Model file for the job. Use its own axes, mm. Face numbers are marked on the shaded views. A direction names the side the tool comes from. Coordinates: 2 decimals unless noted, no trailing zeros. Order: outer loops, then holes, each group sorted by start corner. A loop starts at its lowest first (then second) coordinate and runs counter-clockwise, first axis right, second up.
from build123d import *

# Parameters (mm, degrees)
SKETCH1_W           = 72
SKETCH1_H           = 26
BOSS_EXTRUDE1_DEPTH = 16
SKETCH2_W           = 40
SKETCH2_H           = 26
BOSS_EXTRUDE2_DEPTH = 69
SKETCH3_R           = 3.5
SKETCH3_R_2         = 3
CUT_EXTRUDE1_DEPTH  = 96.5
SKETCH4_R           = 6
CUT_EXTRUDE2_DEPTH  = 6
SKETCH5_R           = 2.5
CUT_EXTRUDE3_DEPTH  = 15


with BuildPart() as part:
    # Sketch1 → Boss-Extrude1 (new body)
    with BuildSketch(Plane(origin=(0, 0, 0), x_dir=(1, 0, 0), z_dir=(0, 1, 0))):
        Rectangle(SKETCH1_W, SKETCH1_H)
    extrude(amount=BOSS_EXTRUDE1_DEPTH)

    # Sketch2 → Boss-Extrude2 (add)
    with BuildSketch(Plane(origin=(0, 16, 0), x_dir=(1, 0, 0), z_dir=(0, 1, 0))):
        Rectangle(SKETCH2_W, SKETCH2_H)
    extrude(amount=BOSS_EXTRUDE2_DEPTH)

    # Sketch3 → Cut-Extrude1 (cut)
    with BuildSketch(Plane(origin=(0, 16, 0), x_dir=(1, 0, 0), z_dir=(0, 1, 0))):
        with Locations(Location((28, 6, 0), (0, 0, 270))):
            Circle(SKETCH3_R)
        with Locations(Location((28, -6, 0), (0, 0, 270))):
            Circle(SKETCH3_R_2)
        with Locations(Location((-28, -6, 0), (0, 0, 270))):
            Circle(SKETCH3_R)
        with Locations(Location((-28, 6, 0), (0, 0, 270))):
            Circle(SKETCH3_R_2)
    extrude(amount=-CUT_EXTRUDE1_DEPTH, mode=Mode.SUBTRACT)

    # Sketch4 → Cut-Extrude2 (cut)
    with BuildSketch(Plane(origin=(0, 16, 0), x_dir=(1, 0, 0), z_dir=(0, 1, 0))):
        with Locations(Location((28, 6, 0), (0, 0, 270))):
            Circle(SKETCH4_R)
        with Locations(Location((-28, -6, 0), (0, 0, 270))):
            Circle(SKETCH4_R)
    extrude(amount=-CUT_EXTRUDE2_DEPTH, mode=Mode.SUBTRACT)

    # Sketch5 → Cut-Extrude3 (cut)
    with BuildSketch(Plane(origin=(0, 85, 0), x_dir=(1, 0, 0), z_dir=(0, 1, 0))):
        with Locations(Location((-3, 5, 0), (0, 0, 270))):
            Circle(SKETCH5_R)
        with Locations(Location((11, 5, 0), (0, 0, 270))):
            Circle(SKETCH5_R)
        with Locations(Location((11, -5, 0), (0, 0, 270))):
            Circle(SKETCH5_R)
        with Locations(Location((-3, -5, 0), (0, 0, 270))):
            Circle(SKETCH5_R)
    extrude(amount=-CUT_EXTRUDE3_DEPTH, mode=Mode.SUBTRACT)


solid = part.part
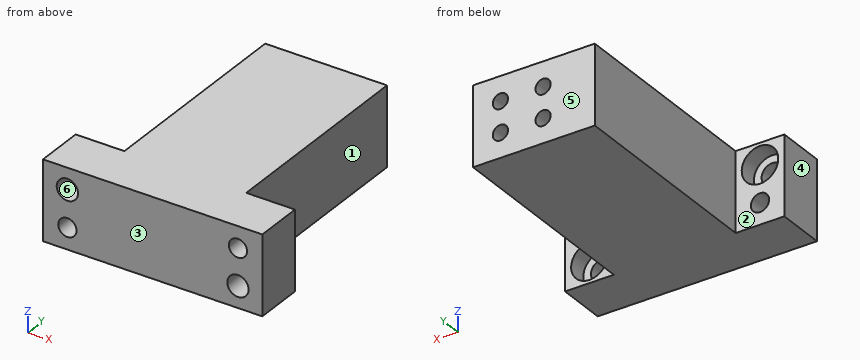
Q1. Cut at C-C, the plane z = -6. List the corners of the cut face in (x, y), plus the area to 3 significant figures.
Established:
outline: (-36, 0) - (-31, 0) - (-31, 16) - (-36, 16) - close; (-25, 0) - (24.5, 0) - (24.5, 10) - (22, 10) - (22, 16) - (20, 16) - (20, 85) - (13.29, 85) - (13.29, 70) - (8.71, 70) - (8.71, 85) - (-0.71, 85) - (-0.71, 70) - (-5.29, 70) - (-5.29, 85) - (-20, 85) - (-20, 16) - (-25, 16) - close; (31.5, 0) - (36, 0) - (36, 16) - (34, 16) - (34, 10) - (31.5, 10) - close
area: 3,540 mm2
Q2. Cut at B-B, the plane x = -28. List the corners of the cut face in (y, z).
Established:
outline: (0, -13) - (16, -13) - (16, -9) - (0, -9) - close; (0, -3) - (16, -3) - (16, 0) - (10, 0) - (10, 2.5) - (0, 2.5) - close; (0, 9.5) - (10, 9.5) - (10, 12) - (16, 12) - (16, 13) - (0, 13) - close
Q3. Drop flat-ended pins along their axis: P1, Ø2.5, axis at x = 11.5, z = 5, coming from the +Y side; P2, Ø14, axis at x = -28, z = 6, coming from the -Y side; P3, Ø12, axis at x = -28, y = 29.5, coming from the -Z side; P4, Ø5, axis at y = 68, z = -8.5, coming from the +X side. Give the stop position or say it passes through.
Established:
P1: stops at y = 70
P2: stops at y = 0
P3: passes through
P4: stops at x = 20
Q4. Probe line 1 (X direction, y = 7, z = 6); line 2 (X direction, y = 80.75, z = 5); line 3 (Y direction, x = 30, z = -2.75). List the from-to ranges inside material, lowest first.
Established:
line 1: x = -36 to -31.5, -24.5 to 25, 31 to 36
line 2: x = -20 to -5.5, -0.5 to 8.5, 13.5 to 20
line 3: y = 0 to 10
Q5. Mould opens along X. For the marked faces 4, 5 and 6 say: pulls with the +X half, pulls with the -X half, needs draft (parallel to the pull), parting line crosses it, or undercut.
Established:
face 4: pulls with the -X half
face 5: needs draft
face 6: undercut
Q6. Which spindle directions (+Z, -Z, +X, -X, +Y, -Y) get a long thin tool onto all of the face, cutting with end or side? Do the marked faces 1, 2 and 3. Say none if no direction does.
Established:
face 1: +Z, -Z, +X, +Y
face 2: +Z, -Z, -X, +Y
face 3: +Z, -Z, +X, -X, -Y
Q7. Cut at A-A, the plane y = 76.5. List the corners of the cut face in (x, z).
Established:
outline: (-20, -13) - (20, -13) - (20, 13) - (-20, 13) - close; hole circle Ø5 at (-3, -5); hole circle Ø5 at (-3, 5); hole circle Ø5 at (11, -5); hole circle Ø5 at (11, 5)
Q8. Cut at D-D, the plane x = -3. List the corners of the cut face in (y, z).
Established:
outline: (0, -13) - (85, -13) - (85, -7.5) - (70, -7.5) - (70, -2.5) - (85, -2.5) - (85, 2.5) - (70, 2.5) - (70, 7.5) - (85, 7.5) - (85, 13) - (0, 13) - close
